Could you check a few things on this model? Use its own coordinates, in mm. Coordinates: 2 decimals unless noted, no trailing zeros. Loops run counter-clockwise (first coordinate to the right, second up) from the corner with the lowest first, then second, coordinate; pieces in that order, holes last.
1) Imagine slicing it at C-C on z = 750. Please give me the cut outline in (x, y), plus the area to 3 significant figures.
2) Will this pin go through, and if not, where does the flat tip stop? P1, Ø1.5, axis at y = 10, z = 274.5, coming from the +X side.
3) Imagine slicing it at A-A on y = 4. Please give me the cut outline in (x, z).
4) If I drill on line 1 along Y through (x, z) = (2.75, 564.5); line 2 along Y through (x, z) = (-9.25, 556), over which ranges is the centre line in solid material (lowest first)?
```python
from build123d import *

# Parameters (mm, degrees)
BOSS_EXTRUDE1_DEPTH = 1094


with BuildPart() as part:
    # Sketch1 → Boss-Extrude1 (new body)
    with BuildSketch(Plane.XY):
        with BuildLine():
            Line((-8.5, -12.5), (8.5, -12.5))
            ThreePointArc((8.5, -12.5), (11.328427125, -11.328427125), (12.5, -8.5))
            Line((12.5, -8.5), (12.5, 8.5))
            ThreePointArc((12.5, 8.5), (11.328427125, 11.328427125), (8.5, 12.5))
            Line((8.5, 12.5), (-8.5, 12.5))
            ThreePointArc((-8.5, 12.5), (-11.328427125, 11.328427125), (-12.5, 8.5))
            Line((-12.5, 8.5), (-12.5, -8.5))
            ThreePointArc((-12.5, -8.5), (-11.328427125, -11.328427125), (-8.5, -12.5))
        make_face()
        with BuildLine():
            Line((-8.5, -10.5), (8.5, -10.5))
            ThreePointArc((8.5, -10.5), (9.914213562, -9.914213562), (10.5, -8.5))
            Line((10.5, -8.5), (10.5, 8.5))
            ThreePointArc((10.5, 8.5), (9.914213562, 9.914213562), (8.5, 10.5))
            Line((8.5, 10.5), (-8.5, 10.5))
            ThreePointArc((-8.5, 10.5), (-9.914213562, 9.914213562), (-10.5, 8.5))
            Line((-10.5, 8.5), (-10.5, -8.5))
            ThreePointArc((-10.5, -8.5), (-9.914213562, -9.914213562), (-8.5, -10.5))
        make_face(mode=Mode.SUBTRACT)
    extrude(amount=BOSS_EXTRUDE1_DEPTH)


solid = part.part
```
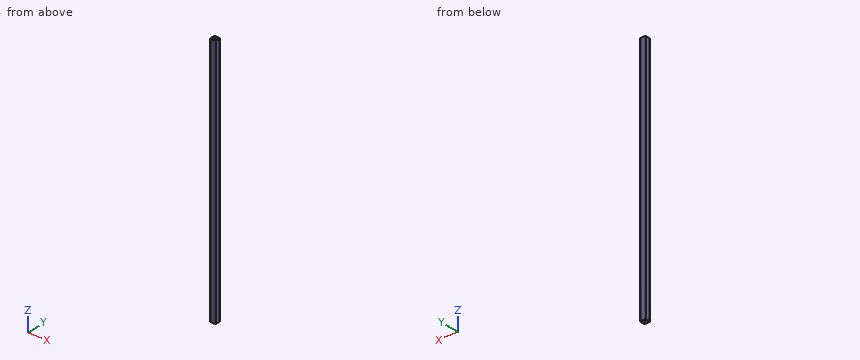
Filled in:
1. outline: (-12.5, -8.5) arc R4 ccw to (-8.5, -12.5) - (8.5, -12.5) arc R4 ccw to (12.5, -8.5) - (12.5, 8.5) arc R4 ccw to (8.5, 12.5) - (-8.5, 12.5) arc R4 ccw to (-12.5, 8.5) - close; hole (-10.5, -8.5) arc R2 ccw to (-8.5, -10.5) - (8.5, -10.5) arc R2 ccw to (10.5, -8.5) - (10.5, 8.5) arc R2 ccw to (8.5, 10.5) - (-8.5, 10.5) arc R2 ccw to (-10.5, 8.5) - close
1. area: 174 mm2
2. P1: stops at x = 12.43
3. outline: (-12.5, 0) - (-10.5, 0) - (-10.5, 1094) - (-12.5, 1094) - close; (10.5, 0) - (12.5, 0) - (12.5, 1094) - (10.5, 1094) - close
4. line 1: y = -12.5 to -10.5, 10.5 to 12.5
4. line 2: y = -12.43 to -10.35, 10.35 to 12.43
